from build123d import *

# Parameters (mm, degrees)
BRACKET_SIDE_PROFILE_SKETCH_R    = 9
BRACKET_SIDE_PROFILE_SKETCH_R_2  = 5
BRACKET_BODY_60MM_DEPTH          = 30
BODY_FILLETS_RADIUS              = 30
BODY_FILLETS_LENGTH              = 12
BORE_13_DEPTH                    = 12
CLEVIS_SLOT_REACH                = 102.001
CLEVIS_SLOT_SKETCH_W             = 45
CLEVIS_SLOT_SKETCH_H             = 40
SADDLE_CUT_REACH                 = 74.139
SADDLE_CUT_SKETCH_R              = 9
SADDLE_CUT_SKETCH_R_2            = 8
BASE_UNDERSIDE_RELIEF_REACH      = 96.129
BASE_UNDERSIDE_RELIEF_END_RADIUS = 30
BASE_UNDERSIDE_RELIEF_SKETCH_W   = 40
BASE_UNDERSIDE_RELIEF_SKETCH_H   = 6


with BuildPart() as part:
    # Bracket Side Profile Sketch → Bracket Body 60mm (new, symmetric)
    with BuildSketch(Plane(origin=(0, 0, 0), x_dir=(0, 0, -1), z_dir=(1, 0, 0))):
        with BuildLine():
            Line((0, 12), (0, 25))
            Line((0, 25), (12, 25))
            Line((12, 25), (12, 52.5))
            ThreePointArc((12, 52.5), (42, 69.820508076), (42, 35.179491924))
            Line((42, 35.179491924), (42, 6))
            Line((42, 6), (50, 6))
            Line((50, 6), (50, 0))
            Line((50, 0), (-50, 0))
            Line((-50, 0), (-50, 12))
            Line((-50, 12), (0, 12))
        make_face()
        with Locations((32, 52.5)):
            Circle(BRACKET_SIDE_PROFILE_SKETCH_R, mode=Mode.SUBTRACT)
        with Locations((27, 12)):
            Circle(BRACKET_SIDE_PROFILE_SKETCH_R_2, mode=Mode.SUBTRACT)
    extrude(amount=BRACKET_BODY_60MM_DEPTH, both=True)

    # Body Fillets: full round fillet: the end face becomes a half cylinder, R = half its width
    body_fillets_face = Plane((0, 6, 50), x_dir=(0, -1, 0), z_dir=(0, 0, 1))  # on the end face: x along it, z out of the body
    body_fillets_slab = body_fillets_face.offset(-BODY_FILLETS_RADIUS / 2) * Box(BODY_FILLETS_LENGTH, 2 * BODY_FILLETS_RADIUS, BODY_FILLETS_RADIUS, mode=Mode.PRIVATE)  # the body's end, R deep
    body_fillets_round = Plane((0, 6, 20), x_dir=(0, 0, 1), z_dir=(0, -1, 0)) * Cylinder(BODY_FILLETS_RADIUS, BODY_FILLETS_LENGTH, mode=Mode.PRIVATE)  # its axis R under the face
    add(body_fillets_slab - body_fillets_round, mode=Mode.SUBTRACT)

    # Bore _13 Sketch → Bore _13 (cut)
    with BuildSketch(Plane.XY):
        with BuildLine():
            Line((-13, 25), (13, 25))
            ThreePointArc((13, 25), (0, 12), (-13, 25))
        make_face()
    extrude(amount=-BORE_13_DEPTH, mode=Mode.SUBTRACT)

    # Clevis Slot Sketch → Clevis Slot (cut, up to next)
    with BuildSketch(Plane.XY.offset(-12), mode=Mode.PRIVATE) as clevis_slot_sk1:
        with Locations((0, 52.5)):
            Rectangle(CLEVIS_SLOT_SKETCH_W, CLEVIS_SLOT_SKETCH_H)
    clevis_slot_tool1 = extrude(clevis_slot_sk1.sketch, amount=-CLEVIS_SLOT_REACH, mode=Mode.PRIVATE) & part.part
    add(clevis_slot_tool1.solids().sort_by_distance((0, 52.5, -12))[0], mode=Mode.SUBTRACT)

    # Saddle Cut: up to this face of the body (flat: up to its plane)
    saddle_cut_end = Plane(part.part.faces().sort_by_distance((0, 0, -2.979428252))[0])
    # Saddle Cut Sketch → Saddle Cut (cut, up to the picked face)
    with BuildSketch(Plane(origin=(0, 32.5, 0), x_dir=(1, 0, 0), z_dir=(0, 1, 0)), mode=Mode.PRIVATE) as saddle_cut_sk1:
        with Locations(Location((0, 27, 0), (0, 0, 180))):
            Circle(SADDLE_CUT_SKETCH_R)
    saddle_cut_tool1 = split(extrude(saddle_cut_sk1.sketch, amount=-SADDLE_CUT_REACH, mode=Mode.PRIVATE), bisect_by=saddle_cut_end, keep=Keep.BOTH, mode=Mode.PRIVATE)
    # Saddle Cut Sketch → Saddle Cut (cut, up to the picked face)
    with BuildSketch(Plane(origin=(0, 32.5, 0), x_dir=(1, 0, 0), z_dir=(0, 1, 0)), mode=Mode.PRIVATE) as saddle_cut_sk2:
        with Locations(Location((0, -20, 0), (0, 0, 270))):
            Circle(SADDLE_CUT_SKETCH_R_2)
    saddle_cut_tool2 = split(extrude(saddle_cut_sk2.sketch, amount=-SADDLE_CUT_REACH, mode=Mode.PRIVATE), bisect_by=saddle_cut_end, keep=Keep.BOTH, mode=Mode.PRIVATE)
    add(saddle_cut_tool1.solids().sort_by(Axis((0, 32.5, -27), (0, -1, 0)))[0], mode=Mode.SUBTRACT)
    add(saddle_cut_tool2.solids().sort_by(Axis((0, 32.5, 20), (0, -1, 0)))[0], mode=Mode.SUBTRACT)

    # Base Underside Relief: up to this cylinder (the profile starts inside it)
    base_underside_relief_end = Plane(origin=(0, 3, 20), z_dir=(0, -1, 0)) * Cylinder(BASE_UNDERSIDE_RELIEF_END_RADIUS, 253.258, mode=Mode.PRIVATE)
    # Base Underside Relief Sketch → Base Underside Relief (cut, up to the surface)
    with BuildSketch(Plane.XY, mode=Mode.PRIVATE) as base_underside_relief_sk1:
        with Locations((0, 3)):
            Rectangle(BASE_UNDERSIDE_RELIEF_SKETCH_W, BASE_UNDERSIDE_RELIEF_SKETCH_H)
    base_underside_relief_tool1 = extrude(base_underside_relief_sk1.sketch, amount=BASE_UNDERSIDE_RELIEF_REACH, mode=Mode.PRIVATE) & base_underside_relief_end
    add(base_underside_relief_tool1.solids().sort_by_distance((0, 3, 0))[0], mode=Mode.SUBTRACT)


solid = part.part
Input: part model. Units: mm. Frame: model coordinates. A direction names the side the tool comes from. Give positions to 0.01 mm unless a question says otherwise; leave off trailing zeros. Order: outer loops, then holes, each group sorted by start corner. A loop starts at its lowest first (then second) coordinate and runs counter-clockwise, first axis right, second up. Notation, with made-up numbers: (39, 74.25) - (52, 74.25) arc R20 cw to (52, 80.25) - close; hole circle Ø6 at (11, 29). An arc over 180 degrees is marked (long way). Write each question's results on one line, items separated by ' | '.
Item 1: Material intervals for line 1 along Z through (x, y) = (-28, 52); line 2 along X through (y, z) = (25.5, -27); line 3 along X through (y, z) = (40.5, -26.5), sorted ascending.
A:
line 1: z = -51.99 to -40.99, -23.01 to -12 | line 2: x = -30 to -9, 9 to 30 | line 3: x = -30 to -22.5, 22.5 to 30
Item 2: Section C-C (y = 46). Return loops of the section in (x, z).
A:
outline: (-30, -50.91) - (-22.5, -50.91) - (-22.5, -38.22) - (-30, -38.22) - close; (-30, -25.78) - (-22.5, -25.78) - (-22.5, -12) - (-30, -12) - close; (22.5, -50.91) - (30, -50.91) - (30, -38.22) - (22.5, -38.22) - close; (22.5, -25.78) - (30, -25.78) - (30, -12) - (22.5, -12) - close
Item 3: Section B-B (z = -25). Return loops of the section in (x, y) (3 decimals).
A:
outline: (-30, 0) - (-8.775, 0) - (-8.775, 7.417) - (-30, 7.417) - close; (-30, 16.583) - (-8.775, 16.583) - (-8.775, 32.5) - (-22.5, 32.5) - (-22.5, 46.843) - (-30, 46.843) - close; (-30, 58.157) - (-22.5, 58.157) - (-22.5, 71.235) - (-30, 71.235) - close; (8.775, 0) - (30, 0) - (30, 7.417) - (8.775, 7.417) - close; (8.775, 16.583) - (30, 16.583) - (30, 46.843) - (22.5, 46.843) - (22.5, 32.5) - (8.775, 32.5) - close; (22.5, 58.157) - (30, 58.157) - (30, 71.235) - (22.5, 71.235) - close
Item 4: Section A-A (x = 5). Return loops of the section in (y, z) (3 decimals), and give its area (3 significant figures).
A:
outline: (0, -50) - (6, -50) - (6, -42) - (32.5, -42) - (32.5, -34.483) - (0, -34.483) - close; (0, -19.517) - (32.5, -19.517) - (32.5, -12) - (13, -12) - (13, 0) - (12, 0) - (12, 13.755) - (6, 13.755) - (6, 0) - (0, 0) - close; (6, 26.245) - (12, 26.245) - (12, 49.58) - (6, 49.58) - close | area: 915 mm^2
Item 5: Draft query along X for faces 4 (the flat face through (0, 0, -15)), 5 (the flat face through (-20, 3, 21)). Return one class per face: released by +X, released by -X, zero draft, split by the parting line, or undercut.
A:
face 4: zero draft | face 5: undercut
Item 6: Access query for faces 1 (the flat face through (0, 29, -12)), 2 (the flat face through (19, 18, 0)), 3 (the flat face through (20, 3, 21)). Directions: +Z, -Z, +X, -X, +Y, -Y. A direction counts if a zero-diameter tool reaches every point of the face in a straight line with its end or side. Return the directions, or none.
A:
face 1: +Z, +Y | face 2: +Z, +X, -X, +Y | face 3: +Z, -Y
Item 7: Contact query for flat-ended pins moving along their axis: pin 1 Ø1.5 at (x, y) = (-20.5, 27.5) entering from +Z; pin 2 Ø5 at (x, y) = (-1, 3) entering from +Z; pin 3 Ø9 at (y, z) = (12, -27) entering from +X; pin 4 Ø15 at (x, z) = (-6, -31) entering from +Y. Output: stop coordinate, or through.
A:
pin 1: stops at z = -12 | pin 2: stops at z = 0 | pin 3: passes through | pin 4: stops at y = 32.5
Item 8: Section D-D (z = 22). Return loops of the section in (x, y), and give its area (3 significant figures).
A:
outline: (-29.93, 0) - (-20, 0) - (-20, 6) - (-7.75, 6) - (-7.75, 12) - (-29.93, 12) - close; (7.75, 6) - (20, 6) - (20, 0) - (29.93, 0) - (29.93, 12) - (7.75, 12) - close | area: 385 mm^2
